from build123d import *

# Parameters (mm, degrees)
SKETCH1_R              = 55
BOSS_EXTRUDE1_DEPTH    = 20
SKETCH2_R              = 4
CUT_EXTRUDE1_DEPTH     = 3
M10_TAPPED_HOLE1_D     = 8.5
M10_TAPPED_HOLE1_DEPTH = 15.23
M10_TAPPED_HOLE1_TIP   = 2.553657631
CHAMFER1_SIZE          = 1


with BuildPart() as part:
    # Sketch1 → Boss-Extrude1 (new body)
    with BuildSketch(Plane(origin=(0, 0, 0), x_dir=(1, 0, 0), z_dir=(0, 1, 0))):
        with BuildLine():
            Line((-47, 63), (47, 63))
            ThreePointArc((47, 63), (58.313708499, 58.313708499), (63, 47))
            Line((63, 47), (63, -47))
            ThreePointArc((63, -47), (58.313708499, -58.313708499), (47, -63))
            Line((47, -63), (-47, -63))
            ThreePointArc((-47, -63), (-58.313708499, -58.313708499), (-63, -47))
            Line((-63, -47), (-63, 47))
            ThreePointArc((-63, 47), (-58.313708499, 58.313708499), (-47, 63))
        make_face()
        with Locations(Location((0, 0, 0), (0, 0, 270))):
            Circle(SKETCH1_R, mode=Mode.SUBTRACT)
    extrude(amount=BOSS_EXTRUDE1_DEPTH)

    # Sketch2 → Cut-Extrude1 (cut)
    with BuildSketch(Plane(origin=(0, 20, 0), x_dir=(1, 0, 0), z_dir=(0, 1, 0))):
        with Locations(Location((-47, 47, 0), (0, 0, 270))):
            Circle(SKETCH2_R)
        with Locations(Location((47, 47, 0), (0, 0, 270))):
            Circle(SKETCH2_R)
        with Locations(Location((47, -47, 0), (0, 0, 270))):
            Circle(SKETCH2_R)
        with Locations(Location((-47, -47, 0), (0, 0, 270))):
            Circle(SKETCH2_R)
    extrude(amount=-CUT_EXTRUDE1_DEPTH, mode=Mode.SUBTRACT)

    # M10 Tapped Hole1
    with Locations(Plane(origin=(0, 20, 0), x_dir=(1, 0, 0), z_dir=(0, 1, 0))):
        with Locations((-47, 47), (47, 47), (47, -47), (-47, -47)):
            Hole(M10_TAPPED_HOLE1_D / 2, depth=M10_TAPPED_HOLE1_DEPTH)
            with Locations((0, 0, -(M10_TAPPED_HOLE1_DEPTH + M10_TAPPED_HOLE1_TIP / 2))):  # 118° drill point
                Cone(0, M10_TAPPED_HOLE1_D / 2, M10_TAPPED_HOLE1_TIP, mode=Mode.SUBTRACT)

    # Chamfer1
    chamfer1_edges = [part.edges().sort_by_distance(p)[0] for p in [
        (0, 20, -55),
    ]]
    chamfer(chamfer1_edges, length=CHAMFER1_SIZE)


solid = part.part
Verification items for the finished model (mm, model axes). A direction names the side the tool comes from. Coordinates: 2 decimals unless noted, no trailing zeros. Write each loop counter-clockwise with the first axis right and the second up, starting at its lowest first coordinate (ties: lowest second). Pieces come first, ordered by that corner, then holes. Notation, with made-up numbers: (43.25, 4.5) -> (61.25, 4.5) arc R19 ccw to (61.25, 25.5) -> close; hole circle Ø8 at (88.25, 83). An arc over 180 degrees is marked (long way). One line per item, written item: value. Start each with the question number.
Q1. Cross-section at B-B on y = 15.5. Enter the section's corners in (x, z).
Q2. Mould release check, pull along Z, two halves, no side actions. Record for faces 3 (the conical face through (46.46, 2.66, 46.5)), 4 (the flat face through (1, 10, 63)), 5 (the cylindrical face through (51.246, 12.278, 46.813)), 6 (the flat face through (-1, 10, -63)): pulls with the +Z half, pulls with the -Z half, needs draft (parallel to the pull), parting line crosses it, or undercut.
Q3. Thickness scan on L1, parallel to X at y = 13.75, z = 47; L2, parallel to X at y = 15.75, z = -49. Record the ranges inside material, lowest first. Write a range as from..to.
Q4. Access from +Z, -Z, +X, -X, +Y, -Y to the whole of each face (thin tool, end or side, straight path). Record for faces 1 (the cylindrical face through (50.37, 12.28, -44.41)), 2 (the cylindrical face through (58.189, 9.86, -58.437)).
Q5. Go/stop test with flat-tipped pins: P1, Ø7.5, axis at x = 47, z = 47, coming from the -Y side; P2, Ø7.5, axis at x = -47, z = -47, coming from the +Y side; P3, Ø7, axis at x = -47, z = 47, coming from the +Y side. Record where each tip stops, or that it passes through.
Q6. Cross-section at A-A on z = 0. Enter the section's corners in (x, y).
Checked values:
1. outline: (-63, -47) arc R16 ccw to (-47, -63) -> (47, -63) arc R16 ccw to (63, -47) -> (63, 47) arc R16 ccw to (47, 63) -> (-47, 63) arc R16 ccw to (-63, 47) -> close; hole circle Ø110 at (0, 0); hole circle Ø8.5 at (-47, -47); hole circle Ø8.5 at (-47, 47); hole circle Ø8.5 at (47, -47); hole circle Ø8.5 at (47, 47)
2. face 3: undercut
2. face 4: pulls with the +Z half
2. face 5: undercut
2. face 6: pulls with the -Z half
3. L1: x = -63..-51.25, -42.75..-28.57, 28.57..42.75, 51.25..63
3. L2: x = -62.87..-50.75, -43.25..-24.98, 24.98..43.25, 50.75..62.87
4. face 1: +Y
4. face 2: -Z, +X, +Y, -Y
5. P1: stops at y = 0
5. P2: stops at y = 4.47
5. P3: stops at y = 4.32
6. outline: (-63, 0) -> (-55, 0) -> (-55, 19) -> (-56, 20) -> (-63, 20) -> close; (55, 0) -> (63, 0) -> (63, 20) -> (56, 20) -> (55, 19) -> close
